from build123d import *

# Parameters (mm, degrees)
BASE_BLOCK_SKETCH_W = 32
BASE_BLOCK_SKETCH_H = 12
BASE_BLOCK_DEPTH    = 52
UPRIGHT_BODY_DEPTH  = 52
CLEVIS_LUG_SKETCH_R = 5
CLEVIS_LUG_DEPTH    = 10
PIVOT_ARM_SKETCH_R  = 8
PIVOT_ARM_DEPTH     = 6


with BuildPart() as part:
    # Base Block Sketch → Base Block (new body)
    with BuildSketch(Plane.XY):
        with Locations((16, 6)):
            Rectangle(BASE_BLOCK_SKETCH_W, BASE_BLOCK_SKETCH_H)
    extrude(amount=BASE_BLOCK_DEPTH)

    # Upright Profile Sketch → Upright Body (add)
    with BuildSketch(Plane.XY.offset(52)):
        Polygon((32, 12), (32, 70), (14, 70), (7, 34), (7, 12), align=None)
    extrude(amount=-UPRIGHT_BODY_DEPTH)

    # Clevis Lug Sketch → Clevis Lug (add)
    with BuildSketch(Plane.XY.offset(6)):
        with BuildLine():
            Line((32, 70), (61, 70))
            ThreePointArc((61, 70), (70.751033946, 62.217506931), (65.324597071, 50.983467397))
            Line((65.324597071, 50.983467397), (32, 35))
            Line((32, 35), (32, 70))
        make_face()
        with Locations((61, 60)):
            Circle(CLEVIS_LUG_SKETCH_R, mode=Mode.SUBTRACT)
    clevis_lug = extrude(amount=CLEVIS_LUG_DEPTH)

    # Clevis Lug Mirror: Clevis Lug across plane
    add(clevis_lug.mirror(Plane.XY.offset(26)))

    # Pivot Arm Sketch → Pivot Arm (add, symmetric)
    with BuildSketch(Plane.XY.offset(26)):
        with BuildLine():
            Line((14, 70), (-24.705108972, 75.115128486))
            ThreePointArc((-24.705108972, 75.115128486), (-42.507231042, 62.306961592), (-30.8017068, 43.761196803))
            Line((-30.8017068, 43.761196803), (7, 34))
            Line((7, 34), (14, 70))
        make_face()
        with Locations((-26.801384807, 59.253047046)):
            Circle(PIVOT_ARM_SKETCH_R, mode=Mode.SUBTRACT)
    extrude(amount=PIVOT_ARM_DEPTH, both=True)


solid = part.part
Read the model definition and answer for the solid it produces. Units are mm, in the model's axes. A direction names the side the tool comes from. Round coordinates to 2 decimals unless told otherwise and drop trailing zeros. Loops run counter-clockwise (first coordinate to the right, second up) from the corner with the lowest first, then second, coordinate; pieces in that order, holes last. Notation, with made-up numbers: (-17, 38) - (21, 38) arc R22 ccw to (21, 75) - close; hole circle Ø1 at (-17, 25.5). An arc over 180 degrees is marked (long way). One line per question, with ' | ' between items. Start each with the question number.
Q1. Flat-ended cylindrical pins translate along their axes: pin 1 (1.5 mm diameter, centred on y = 32.5, z = 33, fed in from +X); pin 2 (3.5 mm diameter, centred on x = 3.5, z = 23.5, fed in from +Y); pin 3 (13 mm diameter, centred on y = 7.5, z = 16, fed in from -X). Find the tip coordinate at first contact, or state that the pin passes through.
Q2. Section C-C on x = 59 is taken. Give the vertices of the cut face in (y, z), plus the area to 3 significant figures.
Q3. Find the intervals of material crossed by L1, parallel to Z at x = 62.5, y = 69.5; L2, parallel to Z at x = -6.5, y = 54; L3, parallel to Y at x = 23.5, z = 36.5, in increasing order.
Q4. For a pull along Y with two mould halves and no side action, classify faces 5 (the flat face through (19, 35, 0)), 6 (the flat face through (7, 23, 26)), 7 (the flat face through (48.896, 43.104, 10.93)), 8 (the flat face through (3, 12, 26)) as +Y half, -Y half, draft (parallel to the pull), parting line (faces both ways), or undercut.
Q5. Section A-A on z = 40 is taken. Give the vertices of the cut face in (x, y).
Q6. Section D-D on y = 42 is taken. Give the vertices of the cut face in (x, z), plus the area to 3 significant figures.
Q7. For faces 1 (the flat face through (0, 6, 26)), 2 (the flat face through (10.55, 52.25, 42.14)), 3 (the flat face through (47, 57, 36)), 4 (the flat face through (47, 57, 6)), determine the directions among +Z, -Z, +X, -X, +Y, -Y from which every point of the face is accessible in a straight line to the end or side of a thin tool.
Q8. Section B-B on x = 42.5 is taken. Give the vertices of the cut face in (y, z), plus the area to 3 significant figures.
Established:
1) pin 1: x = 32 | pin 2: y = 71.62 | pin 3: x = 0
2) outline: (47.95, 6) - (55.42, 6) - (55.42, 16) - (47.95, 16) - close; (47.95, 36) - (55.42, 36) - (55.42, 46) - (47.95, 46) - close; (64.58, 6) - (70, 6) - (70, 16) - (64.58, 16) - close; (64.58, 36) - (70, 36) - (70, 46) - (64.58, 46) - close | area: 258 mm²
3) L1: 6 to 16, 36 to 46 | L2: 20 to 32 | L3: 0 to 70
4) face 5: draft | face 6: undercut | face 7: -Y half | face 8: undercut
5) outline: (0, 0) - (32, 0) - (32, 35) - (65.32, 50.98) arc R10 ccw to (61, 70) - (14, 70) - (7, 34) - (7, 12) - (0, 12) - close; hole circle Ø10 at (61, 60)
6) outline: (-23.98, 20) - (8.56, 20) - (8.56, 0) - (32, 0) - (32, 6) - (46.59, 6) - (46.59, 16) - (32, 16) - (32, 36) - (46.59, 36) - (46.59, 46) - (32, 46) - (32, 52) - (8.56, 52) - (8.56, 32) - (-23.98, 32) - close | area: 1,900 mm²
7) face 1: +Z, -Z, -X, -Y | face 2: +Z, -X, +Y | face 3: +X, +Y, -Y | face 4: -Z, +X, +Y, -Y
8) outline: (40.04, 6) - (70, 6) - (70, 16) - (40.04, 16) - close; (40.04, 36) - (70, 36) - (70, 46) - (40.04, 46) - close | area: 599 mm²
